from build123d import *

# Parameters (mm, degrees)
SKETCH1_W           = 195
SKETCH1_H           = 250
SKETCH1_W_2         = 68
SKETCH1_H_2         = 200
BOSS_EXTRUDE1_DEPTH = 8
F_13_5_HOLE1_D      = 13.5
FILLET2_R           = 20
FILLET3_R           = 10


with BuildPart() as part:
    # Sketch1 → Boss-Extrude1 (new, symmetric)
    with BuildSketch(Plane.XY):
        Rectangle(SKETCH1_W, SKETCH1_H)
        Rectangle(SKETCH1_W_2, SKETCH1_H_2, mode=Mode.SUBTRACT)
    extrude(amount=BOSS_EXTRUDE1_DEPTH, both=True)

    # Ø13.5 Hole1 (through all)
    with Locations(Plane.XY.offset(8)):
        with Locations((-70, 67.5), (70, 67.5), (70, -67.5), (-70, -67.5)):
            Hole(F_13_5_HOLE1_D / 2)

    # Fillet2
    fillet2_edges = [part.edges().sort_by_distance(p)[0] for p in [
        (-97.5, 125, 0),
        (97.5, 125, 0),
        (97.5, -125, 0),
        (-97.5, -125, 0),
    ]]
    fillet(fillet2_edges, radius=FILLET2_R)

    # Fillet3
    fillet3_edges = [part.edges().sort_by_distance(p)[0] for p in [
        (-34, 100, 0),
        (-34, -100, 0),
        (34, -100, 0),
        (34, 100, 0),
    ]]
    fillet(fillet3_edges, radius=FILLET3_R)


solid = part.part
Work out the finished part from the listing and answer in its coordinate system (mm). A direction names the side the tool comes from. Give positions to 0.01 mm unless a question says otherwise; leave off trailing zeros. Loops run counter-clockwise (first coordinate to the right, second up) from the corner with the lowest first, then second, coordinate; pieces in that order, holes last. Notation, with made-up numbers: (-20, 22.5) -> (25, 22.5) arc R22 cw to (25, 40.5) -> close; hole circle Ø2 at (23.5, -21). An arc over 180 degrees is marked (long way). Use a Markdown table: item, result. Add a question column.
1. Find the intervals of material crossed by probe 1 along Y at (x, z) = (70, 2.75); probe 2 along X at (y, z) = (-90, -1); probe 3 along Y at (x, z) = (21, 6), in increasing order.
2. Determine the mould class of faces 3 (the flat face through (0, -100, 0)), 4 (the flat face through (-45, 2, 8)), 5 (the cylindrical face through (91.486, 119.297, -0.112)) for opening direction Y: released by +Y, released by -Y, zero draft, split by the parting line, or undercut.
3. Section A-A on x = -18.5 is taken. Determine the outline of the cut face in (y, z).
4. Section C-C on z = 3.75 is taken. Determine the outline of the cut face in (x, y), and give its area (3 significant figures).
5. For faces 1 (the cylindrical face through (91.486, -119.297, 0.112)), 2 (the cylindrical face through (-31.15, 96.99, -0.11)), determine the directions among +Z, -Z, +X, -X, +Y, -Y from which every point of the face is accessible in a straight line to the end or side of a thin tool.
6. Section D-D on y = -67.5 is taken. Determine the outline of the cut face in (x, z).
7. Section B-B on y = 6 is taken. Determine the outline of the cut face in (x, z), and give its area (3 significant figures).
Results below:
| question | item | result |
|---|---|---|
| 1 | probe 1 | y = -125 to -74.25, -60.75 to 60.75, 74.25 to 125 |
| 1 | probe 2 | x = -97.5 to -34, 34 to 97.5 |
| 1 | probe 3 | y = -125 to -100, 100 to 125 |
| 2 | face 3 | undercut |
| 2 | face 4 | zero draft |
| 2 | face 5 | released by +Y |
| 3 | outline | (-125, -8) -> (-100, -8) -> (-100, 8) -> (-125, 8) -> close; (100, -8) -> (125, -8) -> (125, 8) -> (100, 8) -> close |
| 4 | outline | (-97.5, -105) arc R20 ccw to (-77.5, -125) -> (77.5, -125) arc R20 ccw to (97.5, -105) -> (97.5, 105) arc R20 ccw to (77.5, 125) -> (-77.5, 125) arc R20 ccw to (-97.5, 105) -> close; hole circle Ø13.5 at (-70, -67.5); hole circle Ø13.5 at (-70, 67.5); hole (-34, -90) arc R10 ccw to (-24, -100) -> (24, -100) arc R10 ccw to (34, -90) -> (34, 90) arc R10 ccw to (24, 100) -> (-24, 100) arc R10 ccw to (-34, 90) -> close; hole circle Ø13.5 at (70, -67.5); hole circle Ø13.5 at (70, 67.5) |
| 4 | area | 34,300 mm^2 |
| 5 | face 1 | +Z, -Z, +X, -Y |
| 5 | face 2 | +Z, -Z |
| 6 | outline | (-97.5, -8) -> (-76.75, -8) -> (-76.75, 8) -> (-97.5, 8) -> close; (-63.25, -8) -> (-34, -8) -> (-34, 8) -> (-63.25, 8) -> close; (34, -8) -> (63.25, -8) -> (63.25, 8) -> (34, 8) -> close; (76.75, -8) -> (97.5, -8) -> (97.5, 8) -> (76.75, 8) -> close |
| 7 | outline | (-97.5, -8) -> (-34, -8) -> (-34, 8) -> (-97.5, 8) -> close; (34, -8) -> (97.5, -8) -> (97.5, 8) -> (34, 8) -> close |
| 7 | area | 2,030 mm^2 |
